The listing builds one solid part. Answer for the finished solid, in the listing's coordinates (mm). Face numbers are marked on the shaded views. A direction names the side the tool comes from. Give positions to 0.01 mm unless a question says otherwise; leave off trailing zeros. Order: outer loops, then holes, each group sorted by start corner. A loop starts at its lowest first (then second) coordinate and runs counter-clockwise, first axis right, second up. Notation, with made-up numbers: (-39, 12.25) -> (9, 12.25) arc R21 ccw to (9, 27.25) -> close; hole circle Ø2 at (39.5, 64). An arc over 180 degrees is marked (long way). Answer as a JSON object with one key per item and string values. Group by question number.
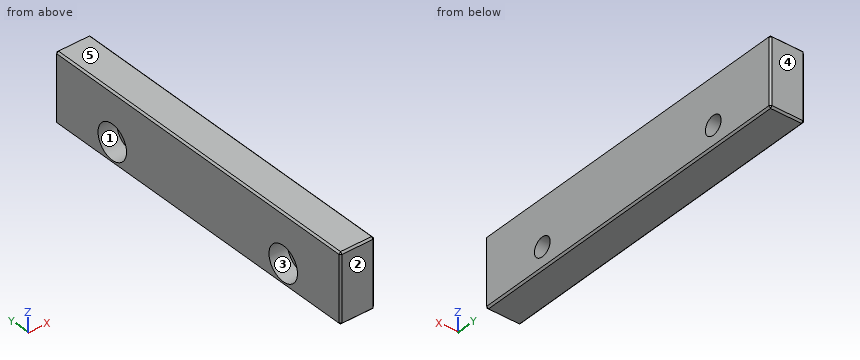
```python
from build123d import *

# Parameters (mm, degrees)
SKETCH_1_W                   = 10
SKETCH_1_H                   = 100
EXTRUDE_1_DEPTH              = 20
HOLE_WIZARD_M5_1_D           = 5.5
HOLE_WIZARD_M5_1_CBORE_D     = 10
HOLE_WIZARD_M5_1_CBORE_DEPTH = 5.4
CHAMFER_1_SIZE               = 0.5


with BuildPart() as part:
    # 草图1 → 凸台-拉伸1 (new body)
    with BuildSketch(Plane.XY):
        Rectangle(SKETCH_1_W, SKETCH_1_H)
    extrude(amount=EXTRUDE_1_DEPTH)

    # M5 六角凹头螺钉的柱形沉头孔1 (through all)
    with Locations(Plane.ZY.offset(5)):
        with Locations((6, 30), (6, -30)):
            CounterBoreHole(HOLE_WIZARD_M5_1_D / 2, HOLE_WIZARD_M5_1_CBORE_D / 2, HOLE_WIZARD_M5_1_CBORE_DEPTH)

    # 倒角1
    chamfer_1_edges = [part.edges().sort_by_distance(p)[0] for p in [
        (-5, 0, 20),
        (0, -50, 20),
        (5, 0, 20),
        (0, -50, 0),
        (-5, 0, 0),
        (0, 50, 0),
        (5, 0, 0),
        (5, -50, 10),
        (-5, -50, 10),
        (-5, 50, 10),
        (5, 50, 10),
        (0, 50, 20),
    ]]
    chamfer(chamfer_1_edges, length=CHAMFER_1_SIZE)


solid = part.part
```
(1) Find the intervals of material crossed by line 1 along Y through (x, z) = (3.15, 6); line 2 along Y through (x, z) = (-1.2, 6), in increasing order. Write a range as [from, to].
(2) A flat-ended cylindrical pin translates along its axis: pin 1 Ø6 at (y, z) = (-30, 6) entering from -X. Find the tip coordinate at first contact, or state that the pin passes through.
(3) A cutting plane is placed at B-B (y = 30). Determine the outline of the cut face in (x, z), and give its area (3 significant figures).
(4) Which of the six approach directions +Z, -Z, +X, -X, +Y, -Y give full straight-line access (tool end or side, diameter ignored) to the marked faces 1 and 2?
(5) For a pull along Z with two mould halves and no side action, classify the marked faces 3, 4 and 5 as +Z half, -Z half, draft (parallel to the pull), parting line (faces both ways), or undercut.
(6) A cutting plane is placed at C-C (x = -0.75). Determine the outline of the cut face in (y, z), and give its area (3 significant figures).
(7) A cutting plane is placed at A-A (z = 6). Determine the outline of the cut face in (x, y), and give its area (3 significant figures).
Check sheet entries:
{
 "1": {"line 1": "y = [-50, -32.75], [-27.25, 27.25], [32.75, 50]", "line 2": "y = [-50, -35], [-25, 25], [35, 50]"},
 "2": {"pin 1": "stops at x = 0.4"},
 "3": {"outline": "(-5, 0.5) -> (-4.5, 0) -> (4.5, 0) -> (5, 0.5) -> (5, 3.25) -> (0.4, 3.25) -> (0.4, 1) -> (-5, 1) -> close; (-5, 11) -> (0.4, 11) -> (0.4, 8.75) -> (5, 8.75) -> (5, 19.5) -> (4.5, 20) -> (-4.5, 20) -> (-5, 19.5) -> close", "area": "120 mm2"},
 "4": {"face 1": "-X", "face 2": "+Z, -Z, +X, -X, -Y"},
 "5": {"face 3": "undercut", "face 4": "draft", "face 5": "+Z half"},
 "6": {"outline": "(-50, 0.5) -> (-49.5, 0) -> (49.5, 0) -> (50, 0.5) -> (50, 19.5) -> (49.5, 20) -> (-49.5, 20) -> (-50, 19.5) -> close; hole circle Ø10 at (-30, 6); hole circle Ø10 at (30, 6)", "area": "1,840 mm2"},
 "7": {"outline": "(-5, -49.5) -> (-4.5, -50) -> (4.5, -50) -> (5, -49.5) -> (5, -32.75) -> (0.4, -32.75) -> (0.4, -35) -> (-5, -35) -> close; (-5, -25) -> (0.4, -25) -> (0.4, -27.25) -> (5, -27.25) -> (5, 27.25) -> (0.4, 27.25) -> (0.4, 25) -> (-5, 25) -> close; (-5, 35) -> (0.4, 35) -> (0.4, 32.75) -> (5, 32.75) -> (5, 49.5) -> (4.5, 50) -> (-4.5, 50) -> (-5, 49.5) -> close", "area": "841 mm2"}
}
